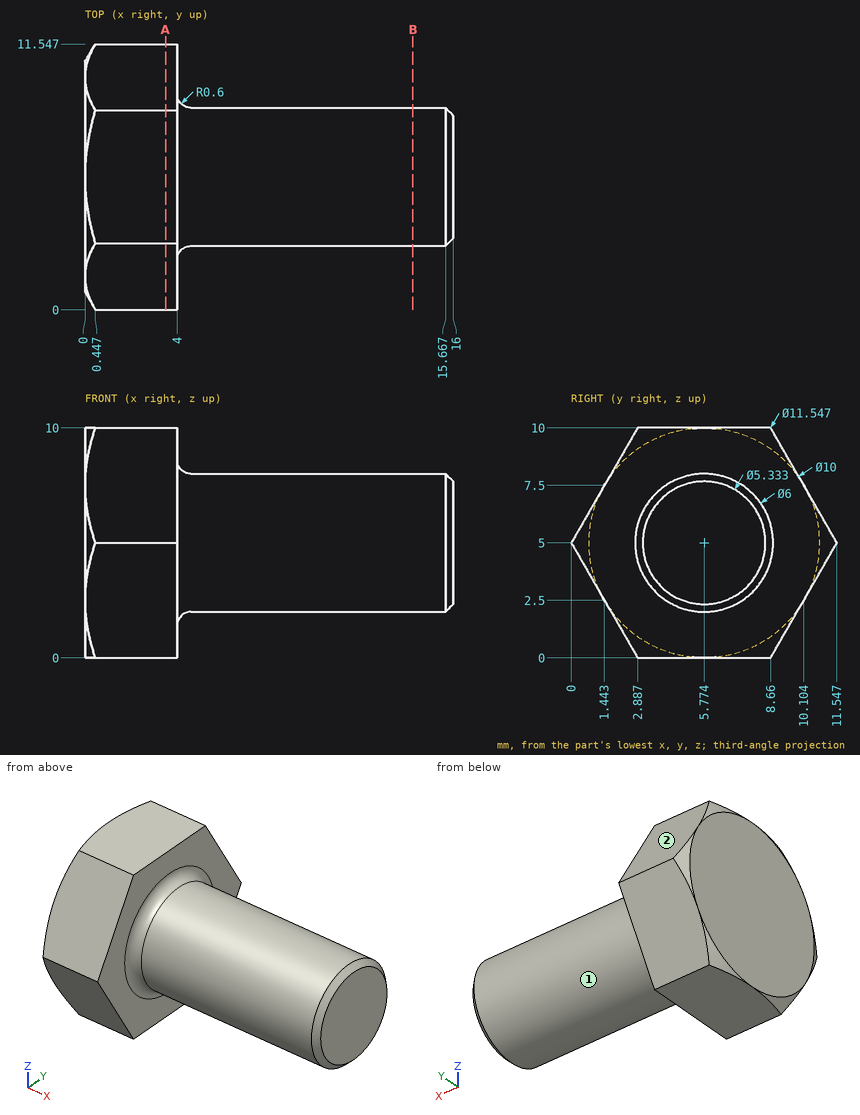
The drawing under review shows one solid part. Ordinate dimensions are in mm from its lowest x, y, z. A direction names the side the tool comes from. Give positions to 0.01 mm unless a question says otherwise; leave off trailing zeros. Order: outer loops, then holes, each group sorted by start corner. A loop starts at its lowest first (then second) coordinate and runs counter-clockwise, first axis right, second up. Notation, with made-up numbers: M 78.5,-25 L 88.5,-25 A20 ccw 88.5,-12 Z; hole C 73,10.5 d6. An arc over 180 degrees is marked long. Answer in a Markdown table with one row per item. Add a question column.
1. To check wall thickness, follow line 1 along X through (y, z) = (10, 7); line 2 along Y through (x, z) = (1, 7.5) (1 decimal); line 3 along Z through (x, y) = (10.5, 7.75) (1 decimal). State the ranges of each line that lie inside material, in increasing order.
2. Add section B-B on x = 14.25. State the section outline as (y, z) points, plus the area to 3 significant figures.
3. Machinability: for the marked faces 1 and 2, which of the approach directions +Z, -Z, +X, -X, +Y, -Y give a long, thin tool a straight path to every point of the face, cutting with its end or side? Answer none if there is none.
4. For pin 1 Ø3 at (x, y) = (6, 2.5) entering from -Z; pin 2 Ø5 at (x, y) = (7.5, 8.5) entering from -Z; pin 3 Ø4 at (x, y) = (14, 2.5) entering from -Z, all flat-tipped, find the tip position at first contact; note any pin that passes through.
5. Add section A-A on x = 3.5. State the section outline as (y, z) points.
The answers:
| question | item | result |
|---|---|---|
| 1 | line 1 | 0 to 4 |
| 1 | line 2 | 1.4 to 10.1 |
| 1 | line 3 | 2.7 to 7.3 |
| 2 | outline | C 5.77,5 d6 |
| 2 | area | 28.3 mm2 |
| 3 | face 1 | +X |
| 3 | face 2 | +Z, +X, -X, +Y |
| 4 | pin 1 | z = 2.58 |
| 4 | pin 2 | z = 2.01 |
| 4 | pin 3 | z = 2.28 |
| 5 | outline | M 0,5 L 2.89,0 L 8.66,0 L 11.55,5 L 8.66,10 L 2.89,10 Z |
